Read the model definition and answer for the solid it produces. Units are mm, in the model's axes. Face numbers are marked on the shaded views. A direction names the side the tool comes from. Coordinates: 2 decimals unless noted, no trailing zeros. Write each loop counter-clockwise with the first axis right and the second up, starting at its lowest first coordinate (ties: lowest second). Pieces come first, ordered by that corner, then holes. Notation, with made-up numbers: (39, 36) -> (96, 36) arc R13 ccw to (96, 45) -> close; hole circle Ø1 at (78, -19.5). An arc over 180 degrees is marked (long way). One line per item, written item: value. Start each with the question number.
1. Find section A-A, the plane y = 0. State how many separate pieces and enclosed holes the cut face has, and give its area (3 significant figures).
2. For the marked faces 1 and 2, determine the directions among +Z, -Z, +X, -X, +Y, -Y from which every point of the face is accessible in a straight line to the end or side of a thin tool.
3. Given P1, Ø4, axis at x = 21.5, z = -26, coming from the -Y side; P2, Ø7, axis at y = 0, z = 35, coming from the +X side; P3, Ø2.5, axis at x = 13, y = 0.5, coming from the +Z side; P4, Ø10, axis at x = 23, z = -21, coming from the -Y side, each flat-ended and moving along its own axis, determine where each tip first touches the part or whether it passes through.
4. Consider line 1 along Y through (x, z) = (23, 0); line 2 along Y through (x, z) = (7.25, 0); line 3 along Z through (x, y) = (18, 2). Determine where each line is inside the solid, lowest interval first.
5. Find section B-B, the plane x = 2.5. Write down the section's boundary in (y, z).
```python
from build123d import *

# Parameters (mm, degrees)
CHAMFER1_SIZE      = 1
CHAMFER2_SIZE      = 0.5
FILLET1_R          = 5
CHAMFER3_SIZE      = 1
SKETCH2_R          = 4.5
CUT_EXTRUDE1_DEPTH = 20
SKETCH3_W          = 8.058064516
SKETCH3_H          = 8
CUT_EXTRUDE2_DEPTH = 69.443407279


with BuildPart() as part:
    # Sketch1 → Revolve1 (revolve)
    with BuildSketch(Plane.XY, mode=Mode.PRIVATE) as revolve1_sk:
        Polygon((0, 12.5), (0, 21), (17, 21), (17, 43.5), (30, 43.5), (30, 12.5), align=None)
    revolve(revolve1_sk.sketch.rotate(Axis((0, 0, 0), (1, 0, 0)), 90), axis=Axis((0, 0, 0), (1, 0, 0)))

    # Chamfer1
    chamfer1_edges = [part.edges().sort_by_distance(p)[0] for p in [
        (0, 0, -21),
    ]]
    chamfer(chamfer1_edges, length=CHAMFER1_SIZE)

    # Chamfer2
    chamfer2_edges = [part.edges().sort_by_distance(p)[0] for p in [
        (30, 0, -12.5),
        (0, 0, -12.5),
    ]]
    chamfer(chamfer2_edges, length=CHAMFER2_SIZE)

    # Fillet1
    fillet1_edges = [part.edges().sort_by_distance(p)[0] for p in [
        (17, 0, -21),
    ]]
    fillet(fillet1_edges, radius=FILLET1_R)

    # Chamfer3
    chamfer3_edges = [part.edges().sort_by_distance(p)[0] for p in [
        (17, 0, -43.5),
        (30, 0, -43.5),
    ]]
    chamfer(chamfer3_edges, length=CHAMFER3_SIZE)

    # Sketch2 → Cut-Extrude1 (cut)
    with BuildSketch(Plane.ZY.offset(-17)):
        with Locations((-35, 0)):
            Circle(SKETCH2_R)
        with Locations((0, -35)):
            Circle(SKETCH2_R)
        with Locations((0, 35)):
            Circle(SKETCH2_R)
        with Locations((35, 0)):
            Circle(SKETCH2_R)
    extrude(amount=-CUT_EXTRUDE1_DEPTH, mode=Mode.SUBTRACT)

    # Sketch3 → Cut-Extrude2 (cut, through all)
    with BuildSketch(Plane(origin=(30, 0, 0), x_dir=(0, 0, -1), z_dir=(1, 0, 0))):
        with Locations((11.770967742, 0)):
            Rectangle(SKETCH3_W, SKETCH3_H)
    extrude(amount=-CUT_EXTRUDE2_DEPTH, mode=Mode.SUBTRACT)


solid = part.part
```
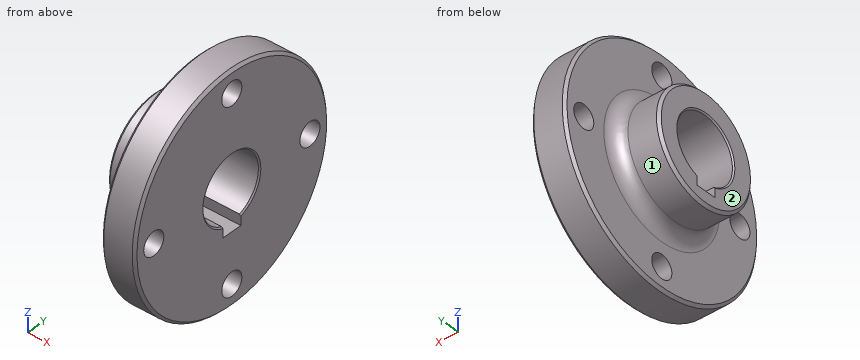
Answer block:
1. separate pieces: 4
1. enclosed holes: 0
1. area: 769 mm2
2. face 1: -X
2. face 2: +Z, -Z, -X, +Y, -Y
3. P1: stops at y = -36.28
3. P2: passes through
3. P3: stops at z = 21.53
3. P4: stops at y = -40.45
4. line 1: y = -43.5 to -39.5, -30.5 to -12.5, 12.5 to 30.5, 39.5 to 43.5
4. line 2: y = -21 to -12.5, 12.5 to 21
4. line 3: z = -43.45 to -39.03, -30.97 to -15.8, 12.34 to 30.97, 39.03 to 43.45
5. outline: circle Ø42 at (0, 0); hole (-4, -15.8) -> (4, -15.8) -> (4, -11.84) arc R12.5 ccw (long way) to (-4, -11.84) -> close
